from build123d import *

# Parameters (mm, degrees)
CLEVIS_LUG_A_SKETCH_R       = 30
CLEVIS_LUG_A_SKETCH_R_2     = 18
CLEVIS_LUG_A_60X_36_DEPTH   = 24
CLEVIS_LUG_B_SKETCH_R       = 30
CLEVIS_LUG_B_SKETCH_R_2     = 18
CLEVIS_LUG_B_60X_36_DEPTH   = 24
ARM_START                   = -18
ARM_WEB_DEPTH               = 18
LUG_START                   = -18
LUG_BRIDGE_DEPTH            = 18
ARM_TOP_PLATE_SKETCH_W      = 54
ARM_TOP_PLATE_SKETCH_H      = 40
ARM_TOP_PLATE_6MM_DEPTH     = 6
ARM_SPINE_SKETCH_R          = 4
ARM_SPINE_54MM_DEPTH        = 54
ARM_BODY_SKETCH_W           = 18
ARM_BODY_SKETCH_H           = 22
ARM_BODY_80MM_DEPTH         = 80
ARM_SIDE_WEB_54MM_DEPTH     = 54
ARM_SLOT_SKETCH_W           = 24
ARM_SLOT_SKETCH_H           = 6
ARM_SLOT_CUT_DEPTH          = 27
ARM_RIB_18MM_REACH          = 137.133
ARM_RIB_SKETCH_WALL_W       = 333.878222312
ARM_RIB_SKETCH_WALL_H       = 18
MOUNTING_FLANGE_SKETCH_R    = 7.5
MOUNTING_FLANGE_DEPTH       = 18
FLANGE_GUSSET_12MM_REACH    = 171.473
FLANGE_GUSSET_SKETCH_WALL_W = 397.51396583
FLANGE_GUSSET_SKETCH_WALL_H = 12


with BuildPart() as part:
    # Clevis Lug A Sketch → Clevis Lug A Ø60xØ36 (new body)
    with BuildSketch(Plane(origin=(0, 0, 0), x_dir=(0, 0, -1), z_dir=(1, 0, 0))):
        Circle(CLEVIS_LUG_A_SKETCH_R)
        Circle(CLEVIS_LUG_A_SKETCH_R_2, mode=Mode.SUBTRACT)
    extrude(amount=CLEVIS_LUG_A_60X_36_DEPTH)

    # Arm Web Sketch → Arm Web (add)
    with BuildSketch(Plane(origin=(18, 0, 0), x_dir=(0, 0, -1), z_dir=(1, 0, 0)).offset(ARM_START)):
        with BuildLine():
            Line((0, 30), (48, 30))
            Line((48, 30), (126, 30))
            Line((126, 30), (126, -4))
            Line((126, -4), (108, -4))
            Line((108, -4), (108, 18))
            Line((108, 18), (48, 18))
            Line((48, 18), (48, -4))
            Line((48, -4), (17.549928775, -4))
            ThreePointArc((17.549928775, -4), (14.071247279, 11.22497216), (0, 18))
            Line((0, 18), (0, 30))
        make_face()
    extrude(amount=ARM_WEB_DEPTH)



with BuildPart() as body_2:
    # Clevis Lug B Sketch → Clevis Lug B Ø60xØ36 (new body)
    with BuildSketch(Plane(origin=(-18, 0, 0), x_dir=(0, 0, -1), z_dir=(1, 0, 0))):
        Circle(CLEVIS_LUG_B_SKETCH_R)
        Circle(CLEVIS_LUG_B_SKETCH_R_2, mode=Mode.SUBTRACT)
    extrude(amount=-CLEVIS_LUG_B_60X_36_DEPTH)

    # Lug Bridge Sketch → Lug Bridge (add)
    with BuildSketch(Plane(origin=(-18, 0, 0), x_dir=(0, 0, -1), z_dir=(1, 0, 0)).offset(LUG_START)):
        with BuildLine():
            Line((0, 30), (126, 30))
            Line((126, 30), (126, -4))
            Line((126, -4), (108, -4))
            Line((108, -4), (108, 18))
            Line((108, 18), (48, 18))
            Line((48, 18), (48, -4))
            Line((48, -4), (17.549928775, -4))
            ThreePointArc((17.549928775, -4), (14.071247279, 11.22497216), (0, 18))
            Line((0, 18), (0, 30))
        make_face()
    extrude(amount=LUG_BRIDGE_DEPTH)


with BuildPart() as part_1:
    add(part.part)

    add(body_2.part)  # Arm Top Plate 6mm merges body 2
    # Arm Top Plate Sketch → Arm Top Plate 6mm (add)
    with BuildSketch(Plane(origin=(0, 30, 0), x_dir=(1, 0, 0), z_dir=(0, 1, 0))):
        with Locations((-9, 106)):
            Rectangle(ARM_TOP_PLATE_SKETCH_W, ARM_TOP_PLATE_SKETCH_H)
    extrude(amount=ARM_TOP_PLATE_6MM_DEPTH)

    # Arm Spine Sketch → Arm Spine 54mm (add)
    with BuildSketch(Plane(origin=(18, 0, 0), x_dir=(0, 0, -1), z_dir=(1, 0, 0))):
        with BuildLine():
            ThreePointArc((24, 18), (29.030770743, 7.564016794), (29.732137495, -4))
            Line((29.732137495, -4), (48, -4))
            Line((48, -4), (48, 18))
            Line((48, 18), (108, 18))
            Line((108, 18), (126, 18))
            Line((126, 18), (126, 30))
            Line((126, 30), (86, 30))
            Line((86, 30), (24, 30))
            Line((24, 30), (24, 18))
        make_face()
        with BuildLine():
            Line((24, 18), (24, -4))
            Line((24, -4), (29.732137495, -4))
            ThreePointArc((29.732137495, -4), (29.030770743, 7.564016794), (24, 18))
        make_face()
        Circle(ARM_SPINE_SKETCH_R)
    extrude(amount=-ARM_SPINE_54MM_DEPTH)


with BuildPart() as arm_spine_54mm_kept_piece:
    # of the separate pieces the step leaves, the one the design keeps (arm_spine_54mm_pieces_kept)
    add(part_1.part.solids().sort_by_distance((-36, 36, -126))[0])

    # Arm Body Sketch → Arm Body 80mm (add)
    with BuildSketch(Plane(origin=(0, 0, -126), x_dir=(-1, 0, 0), z_dir=(0, 0, -1))):
        with Locations((9, 7)):
            Rectangle(ARM_BODY_SKETCH_W, ARM_BODY_SKETCH_H)
    extrude(amount=-ARM_BODY_80MM_DEPTH)

    # Arm Side Web Sketch → Arm Side Web 54mm (add)
    with BuildSketch(Plane(origin=(18, 0, 0), x_dir=(0, 0, -1), z_dir=(1, 0, 0))):
        Polygon((48, -4), (48, -24), (24, -24), (24, 6), (48, 6), align=None)
    extrude(amount=-ARM_SIDE_WEB_54MM_DEPTH)

    # Arm Slot Sketch → Arm Slot Cut (cut, symmetric)
    with BuildSketch(Plane(origin=(-9, 0, 0), x_dir=(0, 0, -1), z_dir=(1, 0, 0))):
        with Locations((36, -21)):
            Rectangle(ARM_SLOT_SKETCH_W, ARM_SLOT_SKETCH_H)
    extrude(amount=ARM_SLOT_CUT_DEPTH, both=True, mode=Mode.SUBTRACT)

    # Arm Rib Sketch wall → Arm Rib 18mm (add, up to next)
    with BuildSketch(Plane(origin=(-9, -11, -78), x_dir=(0, 0.227229615606, -0.973841209742), z_dir=(0, 0.973841209742, 0.227229615606)), mode=Mode.PRIVATE) as arm_rib_18mm_sk1:
        Rectangle(ARM_RIB_SKETCH_WALL_W, ARM_RIB_SKETCH_WALL_H)
    arm_rib_18mm_tool1 = extrude(arm_rib_18mm_sk1.sketch, amount=ARM_RIB_18MM_REACH, mode=Mode.PRIVATE) - arm_spine_54mm_kept_piece.part
    add(arm_rib_18mm_tool1.solids().sort_by_distance((-9, -11, -78))[0])

    # Mounting Flange Sketch → Mounting Flange (add)
    with BuildSketch(Plane(origin=(0, 0, -126), x_dir=(-1, 0, 0), z_dir=(0, 0, -1))):
        with BuildLine():
            Line((-18, 76), (36, 76))
            ThreePointArc((36, 76), (50.142135624, 70.142135624), (56, 56))
            Line((56, 56), (56, -4))
            Line((56, -4), (-38, -4))
            Line((-38, -4), (-38, 56))
            ThreePointArc((-38, 56), (-32.142135624, 70.142135624), (-18, 76))
        make_face()
        with Locations((-18, 56)):
            Circle(MOUNTING_FLANGE_SKETCH_R, mode=Mode.SUBTRACT)
        with Locations((36, 56)):
            Circle(MOUNTING_FLANGE_SKETCH_R, mode=Mode.SUBTRACT)
    extrude(amount=MOUNTING_FLANGE_DEPTH)

    # Flange Gusset Sketch wall → Flange Gusset 12mm (add, up to next)
    with BuildSketch(Plane(origin=(-9, 56, -106), x_dir=(0, 0.707106781187, -0.707106781187), z_dir=(0, 0.707106781187, 0.707106781187)), mode=Mode.PRIVATE) as flange_gusset_12mm_sk1:
        Rectangle(FLANGE_GUSSET_SKETCH_WALL_W, FLANGE_GUSSET_SKETCH_WALL_H)
    flange_gusset_12mm_tool1 = extrude(flange_gusset_12mm_sk1.sketch, amount=-FLANGE_GUSSET_12MM_REACH, mode=Mode.PRIVATE) - arm_spine_54mm_kept_piece.part
    add(flange_gusset_12mm_tool1.solids().sort_by_distance((-9, 56, -106))[0])


solid = arm_spine_54mm_kept_piece.part
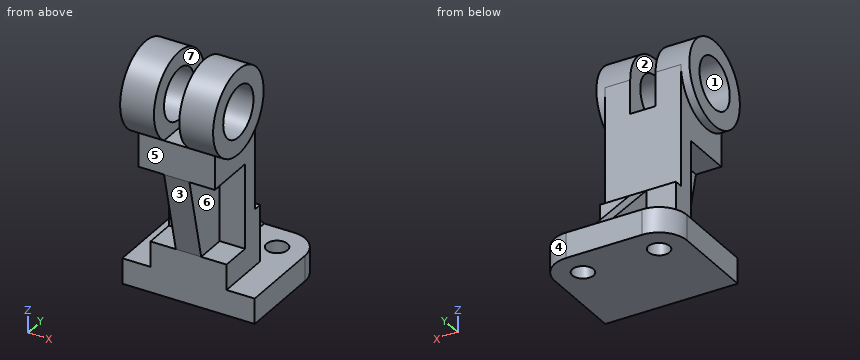
Here's how the part is built. I have some questions about the finished solid (model axes, mm). Face numbers are marked on the shaded views. A direction names the side the tool comes from. Coordinates: 2 decimals unless noted, no trailing zeros. Order: outer loops, then holes, each group sorted by start corner. A loop starts at its lowest first (then second) coordinate and runs counter-clockwise, first axis right, second up.
Item 1: For P1, Ø12, axis at y = -6.5, z = 1.5, coming from the +X side; P2, Ø17, axis at x = -36, y = 56, coming from the +Z side; P3, Ø3, axis at x = 2, z = -8, coming from the +Y side; P4, Ø20.5, axis at x = -30, y = 33, coming from the +Z side, each with a flat end and sliding along its axis, tell me the tip position at first contact or that it passes through.
Result sheet:
P1: passes through
P2: stops at z = -126
P3: stops at y = 30
P4: stops at z = 19.56
Item 2: If we section it at D-D on y = 45.5: List the corners of the cut face in (x, z) for me, plus the area to 3 significant figures.
Result sheet:
outline: (-56, -144) - (38, -144) - (38, -126) - (-3, -126) - (-3, -95.5) - (-15, -95.5) - (-15, -126) - (-56, -126) - close
area: 2,060 mm2
Item 3: For the marked faces 5, 6 and 7, which set-ups out of +Z, -Z, +X, -X, +Y, -Y let a thin tool reach every point of the face, with its end or its side?
Result sheet:
face 5: -Z, +X, -X, -Y
face 6: +X, -Y
face 7: +Z, +Y, -Y
Item 4: If we mould it in two halves opening along Y, with no side actions, what happens to the marked faces 1, 2, 3 and 4? For each: +Y half, -Y half, draft (parallel to the pull), parting line (faces both ways), or undercut.
Result sheet:
face 1: undercut
face 2: draft
face 3: -Y half
face 4: +Y half
Item 5: If we section it at C-C on x = -34: List the corners of the cut face in (y, z) for me, plus the area to 3 significant figures.
Result sheet:
outline: (-18, -48) - (18, -48) - (18, -108) - (-4, -108) - (-4, -144) - (48.77, -144) - (48.77, -126) - (36, -126) - (36, -86) - (30, -86) - (30, 0) arc R30 ccw (long way) to (-18, -24) - close; (63.23, -144) - (76, -144) - (76, -126) - (63.23, -126) - close; hole circle Ø36 at (0, 0)
area: 5,650 mm2
Item 6: If we section it at A-A on y = 0: State how many separate pieces and enclosed holes the cut face has, plus the area to 3 significant figures.
Result sheet:
separate pieces: 3
enclosed holes: 0
area: 5,980 mm2
Item 7: If we section it at B-B on z = -7.5: List the corners of the cut face in (x, y) for me, plus the area to 3 significant figures.
Result sheet:
outline: (-42, -29.05) - (-18, -29.05) - (-18, -16.36) - (-42, -16.36) - close; (-42, 16.36) - (-18, 16.36) - (-18, 30) - (-36, 30) - (-36, 29.05) - (-42, 29.05) - close; (0, -29.05) - (24, -29.05) - (24, -16.36) - (0, -16.36) - close; (0, 16.36) - (24, 16.36) - (24, 29.05) - (18, 29.05) - (18, 30) - (0, 30) - close
area: 1,250 mm2
Item 8: I need wall thicknesses on line 1 (Y direction, x = 18, z = -137); line 2 (Y direction, x = 5, z = 0); line 3 (Z direction, x = 25.5, y = 5.5). Which ranges of each line are inside material? Lowest first, please.
Result sheet:
line 1: y = -4 to 48.5, 63.5 to 76
line 2: y = -30 to -18, 18 to 30
line 3: z = -144 to -126
